Work out the finished part from the listing and answer in its coordinate system (mm). A direction names the side the tool comes from. Give positions to 0.01 mm unless a question says otherwise; leave off trailing zeros. Order: outer loops, then holes, each group sorted by start corner. A loop starts at its lowest first (then second) coordinate and runs counter-clockwise, first axis right, second up. Notation, with made-up numbers: (69, 74.5) -> (96, 74.5) arc R18 ccw to (96, 86.5) -> close; hole circle Ø6 at (24, -32). An arc over 180 degrees is marked (long way). Use a Markdown table: item, result. Add a question column.
```python
from build123d import *

# Parameters (mm, degrees)
BRACKET_PROFILE_SKETCH_R       = 10
BRACKET_PROFILE_SKETCH_R_2     = 6.5
BRACKET_BODY_30_THICK_DEPTH    = 15
SIDE_STEP_CUT_20X10X6_DEPTH    = 6
FORKED_SLOT_15_WIDE_DEPTH      = 93.011635333
FORKED_SLOT_15_WIDE_DEPTH_BACK = 93.011635333
FORK_SLOT_SKETCH_W             = 15
FORK_SLOT_SKETCH_H             = 40


with BuildPart() as part:
    # Bracket Profile Sketch → Bracket Body 30 Thick (new, symmetric)
    with BuildSketch(Plane(origin=(0, 0, 0), x_dir=(0, 0, -1), z_dir=(1, 0, 0))):
        with BuildLine():
            Line((-24.92209858, -1.972055368), (-29.188306629, 51.942687225))
            ThreePointArc((-29.188306629, 51.942687225), (-18.546726282, 67.492876488), (-1.101285774, 60.371905777))
            ThreePointArc((-1.101285774, 60.371905777), (24.520233718, 33.956144929), (60, 24.186760769))
            Line((60, 24.186760769), (60, 11.186760769))
            Line((60, 11.186760769), (35, 11.186760769))
            ThreePointArc((35, 11.186760769), (27.5, 3.686760769), (35, -3.813239231))
            Line((35, -3.813239231), (60, -3.813239231))
            Line((60, -3.813239231), (60, -16.813239231))
            Line((60, -16.813239231), (3.479327524, -24.756701719))
            ThreePointArc((3.479327524, -24.756701719), (-15.643948829, -19.500432432), (-24.92209858, -1.972055368))
        make_face()
        Circle(BRACKET_PROFILE_SKETCH_R, mode=Mode.SUBTRACT)
        with Locations((-14.235047481, 53.125920446)):
            Circle(BRACKET_PROFILE_SKETCH_R_2, mode=Mode.SUBTRACT)
    extrude(amount=BRACKET_BODY_30_THICK_DEPTH, both=True)

    # Side Step Sketch → Side Step Cut 20x10x6 (cut)
    with BuildSketch(Plane(origin=(15, 0, 0), x_dir=(0, 0, -1), z_dir=(1, 0, 0))):
        with BuildLine():
            Line((3.085460595, 43.125920446), (12.306235476, 43.125920446))
            ThreePointArc((12.306235476, 43.125920446), (4.925595155, 51.222687515), (-1.101285774, 60.371905777))
            ThreePointArc((-1.101285774, 60.371905777), (-18.546726282, 67.492876488), (-29.188306629, 51.942687225))
            Line((-29.188306629, 51.942687225), (-28.144793013, 38.755152227))
            ThreePointArc((-28.144793013, 38.755152227), (-11.463003291, 33.318957756), (3.085460595, 43.125920446))
        make_face()
    side_step_cut_20x10x6 = extrude(amount=-SIDE_STEP_CUT_20X10X6_DEPTH, mode=Mode.SUBTRACT)

    # Side Step Cut Mirror: Side Step Cut 20x10x6 across plane
    add(side_step_cut_20x10x6.mirror(Plane(origin=(0, 0, 0), x_dir=(0, 0, 1), z_dir=(1, 0, 0))), mode=Mode.SUBTRACT)

    # Fork Slot Sketch → Forked Slot 15 Wide (cut, two sides: drawn at the far end of the back side and taken through both)
    with BuildSketch(Plane(origin=(0, 0, 0), x_dir=(1, 0, 0), z_dir=(0, 1, 0)).offset(-FORKED_SLOT_15_WIDE_DEPTH_BACK)):
        with Locations((0, 40)):
            Rectangle(FORK_SLOT_SKETCH_W, FORK_SLOT_SKETCH_H)
    extrude(amount=FORKED_SLOT_15_WIDE_DEPTH + FORKED_SLOT_15_WIDE_DEPTH_BACK, mode=Mode.SUBTRACT)


solid = part.part
```
1) The part is cut by section B-B, the plane z = -6.5. Determine the outline of the cut face in (x, y), then the cut area to 3 significant figures.
2) The part is cut by section C-C, the plane x = 2. Determine the outline of the cut face in (y, z), then the cut area to 3 significant figures.
3) Which of the six approach directions +Z, -Z, +X, -X, +Y, -Y give full straight-line access (tool end or side, diameter ignored) to faces 4 (the flat face through (11, -3.813, -47)), 5 (the flat face through (-7.5, 13, -35)), 6 (the cylindrical face through (12.042, 33.285, 11.715)), 7 (the cylindrical face through (-12.042, 33.285, 11.715)), 8 (the flat face through (0.21, -22.495, -19.575))?
4) The part is cut by section A-A, the plane y = 0. Determine the outline of the cut face in (x, z).
5) Flat-ended cylindrical pins translate along their axes: pin 1 (2 mm diameter, centred on x = -11, z = -48.5, fed in from -Y); pin 2 (8 mm diameter, centred on x = 10, z = -37, fed in from -Y); pin 3 (8 mm diameter, centred on x = 13, z = -48, fed in from -Y). Find the tip coordinate at first contact, or state that the pin passes through.
6) Straight lines are drawn through the part: line 1 (Z direction, x = 0, y = 57); line 2 (X direction, y = 53.5, z = -2); line 3 (Y direction, x = -3.5, z = 18.5). For each, find the intervals that lie inside material, in ascending order.
7) Determine the mould class of faces 1 (the flat face through (7.5, 13, -35)), 2 (the flat face through (-11, 11.187, -48)), 3 (the flat face through (-15, 10, -7)) for opening direction X: released by +X, released by -X, zero draft, split by the parting line, or undercut.
8) The part is cut by section D-D, the plane z = -32.5. Determine the outline of the cut face in (x, y), then the cut area to 3 significant figures.
A:
| question | item | result |
|---|---|---|
| 1 | outline | (-15, -24.33) -> (15, -24.33) -> (15, -7.6) -> (-15, -7.6) -> close; (-15, 7.6) -> (15, 7.6) -> (15, 43.13) -> (9, 43.13) -> (9, 49.27) -> (-9, 49.27) -> (-9, 43.13) -> (-15, 43.13) -> close |
| 1 | area | 1,680 mm^2 |
| 2 | outline | (-24.76, -3.48) -> (-22.43, -20) -> (36.87, -20) arc R70 cw to (60.37, 1.1) arc R15 ccw to (51.94, 29.19) -> (-1.97, 24.92) arc R25 ccw to start; hole circle Ø20 at (0, 0); hole circle Ø13 at (53.13, 14.24) |
| 2 | area | 3,240 mm^2 |
| 3 | face 4 | -Z, +X, -X |
| 3 | face 5 | -Z, +Y, -Y |
| 3 | face 6 | +X, +Y |
| 3 | face 7 | -X, +Y |
| 3 | face 8 | -Z, +X, -X, -Y |
| 4 | outline | (-15, -28.47) -> (-7.5, -28.47) -> (-7.5, -20) -> (7.5, -20) -> (7.5, -28.47) -> (15, -28.47) -> (15, -10) -> (-15, -10) -> close; (-15, 10) -> (15, 10) -> (15, 25.08) -> (-15, 25.08) -> close |
| 5 | pin 1 | y = -18.57 |
| 5 | pin 2 | y = -20.61 |
| 5 | pin 3 | y = -19.06 |
| 6 | line 1 | -0.88 to 9.02, 19.45 to 28.73 |
| 6 | line 2 | -9 to 9 |
| 6 | line 3 | -16.82 to 48.22, 58.03 to 67.51 |
| 7 | face 1 | undercut |
| 7 | face 2 | zero draft |
| 7 | face 3 | released by -X |
| 8 | outline | (-15, -20.68) -> (-7.5, -20.68) -> (-7.5, -3.38) -> (-15, -3.38) -> close; (-15, 10.76) -> (-7.5, 10.76) -> (-7.5, 29.9) -> (-15, 29.9) -> close; (7.5, -20.68) -> (15, -20.68) -> (15, -3.38) -> (7.5, -3.38) -> close; (7.5, 10.76) -> (15, 10.76) -> (15, 29.9) -> (7.5, 29.9) -> close |
| 8 | area | 546 mm^2 |
